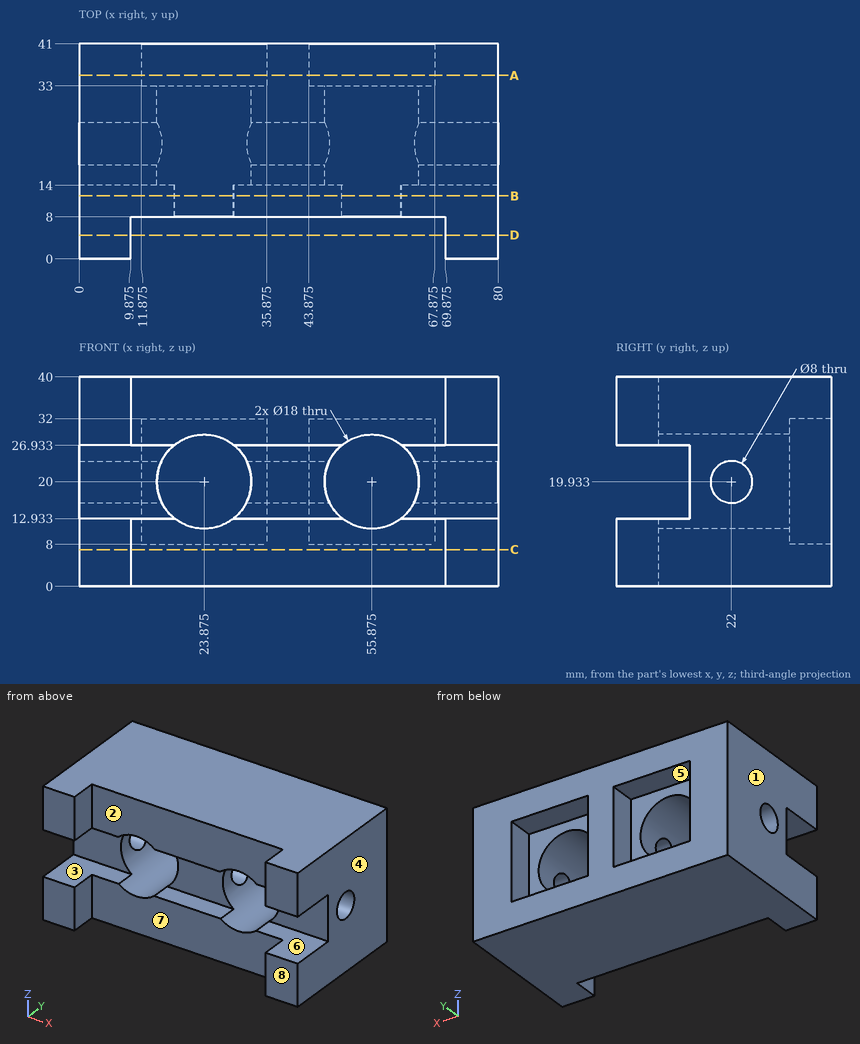
Geometry check sheet. Reference: drawing and pictorial views, mm from the part's lowest x, y, z. A direction names the side the tool comes from. Give positions to 0.01 mm unless a question says otherwise; leave off trailing zeros. Loops run counter-clockwise (first coordinate to the right, second up) from the corner with the lowest first, then second, coordinate; pieces in that order, holes last.
1. Section check D-D, the plane y = 4.5. Enter the section's corners in (x, z) (1 decimal), then the cut area to 3 significant figures.
2. Thickness scan on line 1 (X direction, y = 27.5, z = 20) (1 decimal); line 2 (X direction, y = 3.5, z = 2) (1 decimal); line 3 (Z direction, x = 38, y = 9.5). Record the ranges inside material, lowest first.
3. Section check B-B, the plane y = 12. Enter the section's corners in (x, z) (1 decimal), then the cut area to 3 significant figures.
4. Mould release check, pull along X, two halves, no side actions. Record for the marked faces 1, 2, 3 and 4: released by +X, released by -X, zero draft, split by the parting line, or undercut.
5. Set-up check for the marked faces 5, 6, 7 and 8: record each of +Z, -Z, +X, -X, +Y, -Y from which the full face is reachable in a straight line by a thin tool's end or side.
6. Section check C-C, the plane z = 7. Enter the section's corners in (x, y) (1 decimal), then the cut area to 3 significant figures.
7. Go/stop test with flat-tipped pins: pin 1 Ø8 at (x, z) = (24, 7.5) entering from -Y; pin 2 Ø7 at (x, z) = (70.5, 20.5) entering from -Y. Record where each tip stops, or that it passes through.
8. Section check A-A, the plane y = 35. Enter the section's corners in (x, z) (1 decimal), then the cut area to 3 significant figures.
Geometry says:
1. outline: (0, 0) - (9.9, 0) - (9.9, 12.9) - (0, 12.9) - close; (0, 26.9) - (9.9, 26.9) - (9.9, 40) - (0, 40) - close; (69.9, 0) - (80, 0) - (80, 12.9) - (69.9, 12.9) - close; (69.9, 26.9) - (80, 26.9) - (80, 40) - (69.9, 40) - close
1. area: 520 mm2
2. line 1: x = 0 to 14.9, 32.9 to 46.9, 64.9 to 80
2. line 2: x = 0 to 9.9, 69.9 to 80
2. line 3: z = 0 to 12.93, 26.93 to 40
3. outline: (0, 0) - (80, 0) - (80, 12.9) - (61.4, 12.9) arc R9 cw to (50.3, 12.9) - (29.4, 12.9) arc R9 cw to (18.3, 12.9) - (0, 12.9) - close; (0, 26.9) - (18.1, 26.9) arc R9 cw to (29.6, 26.9) - (50.1, 26.9) arc R9 cw to (61.6, 26.9) - (80, 26.9) - (80, 40) - (0, 40) - close
3. area: 2,020 mm2
4. face 1: released by -X
4. face 2: undercut
4. face 3: zero draft
4. face 4: released by +X
5. face 5: +Y
5. face 6: +X, -X, -Y
5. face 7: +Z, -Z, -Y
5. face 8: +Z, -Z, +X, -X, -Y
6. outline: (0, 0) - (9.9, 0) - (9.9, 8) - (69.9, 8) - (69.9, 0) - (80, 0) - (80, 41) - (0, 41) - close
6. area: 2,800 mm2
7. pin 1: stops at y = 8
7. pin 2: stops at y = 14
8. outline: (0, 0) - (80, 0) - (80, 40) - (0, 40) - close; hole (11.9, 8) - (35.9, 8) - (35.9, 32) - (11.9, 32) - close; hole (43.9, 8) - (67.9, 8) - (67.9, 32) - (43.9, 32) - close
8. area: 2,050 mm2
